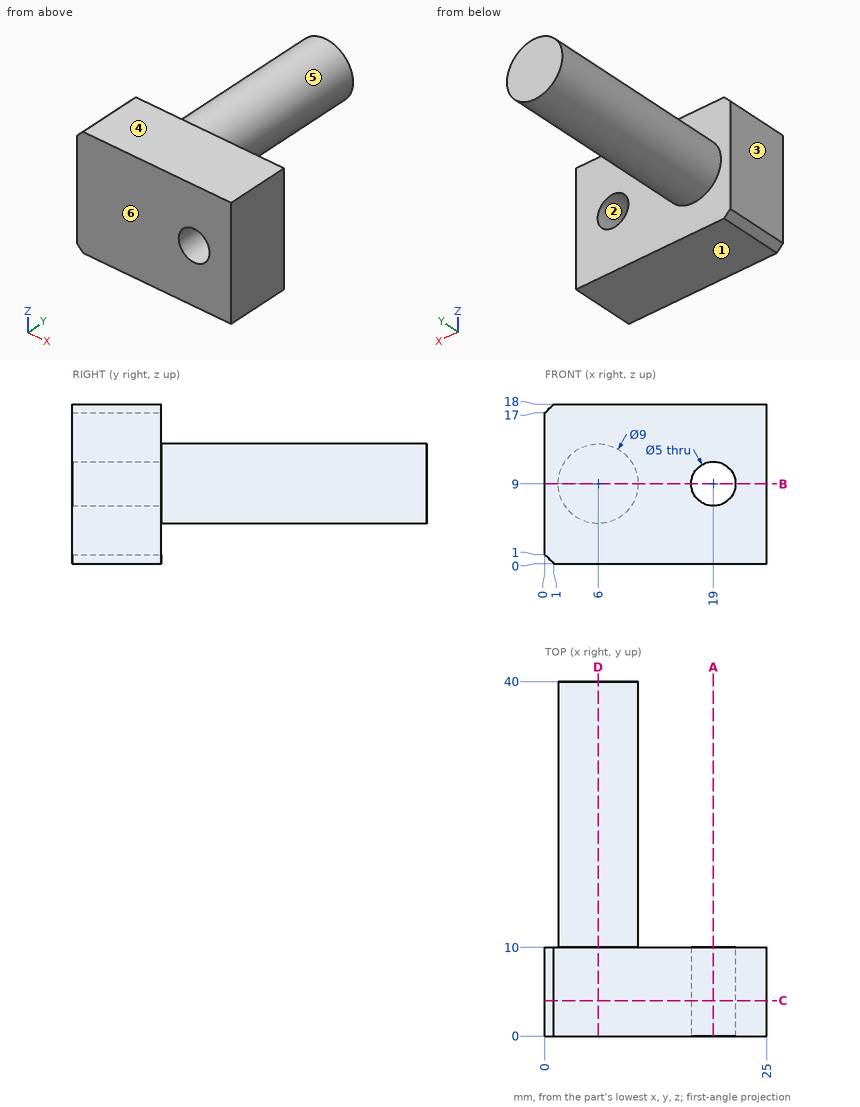
Could you check a few things on this drawing? It's one solid part, dimensions in mm from its lowest x, y, z. A direction names the side the tool comes from. Give positions to 0.01 mm unless a question says otherwise; leave off trailing zeros. Order: outer loops, then holes, each group sorted by start corner. A loop starts at its lowest first (then second) coordinate and runs counter-clockwise, first axis right, second up. Notation, with made-up numbers: M 34.25,7.25 L 86.25,7.25 A13 ccw 86.25,25.25 Z; hole C 61.25,78.5 d5. An arc over 180 degrees is marked long. Use one line per item in the form item = value.
Item 1: Thinking about a two-plate mould opening in Z: for the marked faces 1, 2, 3 and 4, which applies, pulls with the +Z half, pulls with the -Z half, needs draft (parallel to the pull), parting line crosses it, or undercut?
Values follow:
face_1 = pulls with the -Z half
face_2 = undercut
face_3 = needs draft
face_4 = pulls with the +Z half
Item 2: If we section it at B-B, the plane z = 9: Write out the boundary of the cut face in (x, y).
Values follow:
outline = M 0,0 L 16.5,0 L 16.5,10 L 10.5,10 L 10.5,40 L 1.5,40 L 1.5,10 L 0,10 Z; M 21.5,0 L 25,0 L 25,10 L 21.5,10 Z
Item 3: Will these pins go through, and if not, where does the flat tip stop? pin 1 Ø8 at (x, y) = (18, 16) entering from -Z; pin 2 Ø10 at (x, y) = (9.5, 34) entering from -Z; pin 3 Ø1.5 at (x, y) = (9.5, 23) entering from +Z.
Values follow:
pin_1 = through
pin_2 = 4.5
pin_3 = 12.56
Item 4: If we section it at A-A, the plane x = 19: Write out the boundary of the cut face in (y, z).
Values follow:
outline = M 0,0 L 10,0 L 10,6.5 L 0,6.5 Z; M 0,11.5 L 10,11.5 L 10,18 L 0,18 Z
Item 5: If we section it at C-C, the plane y = 4: Write out the boundary of the cut face in (x, z), and give its area (3 significant figures).
Values follow:
outline = M 0,1 L 1,0 L 25,0 L 25,18 L 1,18 L 0,17 Z; hole C 19,9 d5
area = 429 mm^2
Item 6: If I drill on line 1 along Z through (x, y) = (19, 7.25); line 2 along Z through (x, y) = (5.75, 27.5); line 3 along Y through (x, z) = (18.5, 3), over which ranges is the centre line in solid material (lowest first)? Write a range as [from, to].
Values follow:
line_1 = [0, 6.5], [11.5, 18]
line_2 = [4.51, 13.49]
line_3 = [0, 10]
Item 7: If we section it at D-D, the plane x = 6: Write out the boundary of the cut face in (y, z), and give its area (3 significant figures).
Values follow:
outline = M 0,0 L 10,0 L 10,4.5 L 40,4.5 L 40,13.5 L 10,13.5 L 10,18 L 0,18 Z
area = 450 mm^2
Item 8: For the marked faces 5 and 6, which set-ups out of +Z, -Z, +X, -X, +Y, -Y let a thin tool reach every point of the face, with its end or its side?
Values follow:
face_5 = +Y
face_6 = +Z, -Z, +X, -X, -Y
